Verification items for this drawing (mm, ordinates from the low corner). A direction names the side the tool comes from. Round coordinates to 2 decimals unless told otherwise and drop trailing zeros. Order: outer loops, then holes, each group sorted by start corner. A loop starts at its lowest first (then second) coordinate and runs counter-clockwise, first axis right, second up. Notation, with made-up numbers: (-35, 16.25) -> (10, 16.25) arc R18 cw to (10, 43.25) -> close; hole circle Ø4 at (59.25, 84). An arc over 180 degrees is marked (long way). Answer in a Markdown table with one row per item. Add a question column.
1. Material ranges on L1, parallel to Y at x = 14, z = 6; L2, parallel to Y at x = 13, z = 9.5; L3, parallel to Z at x = 22.5, y = 58, recorded low to high. Write a range as from..to.
2. Sectioned sample at C-C, the plane x = 35.5. Record the boundary of the cut face in (y, z).
3. Access from +Z, -Z, +X, -X, +Y, -Y to the whole of each face (thin tool, end or side, straight path). Record for the marked faces 1, 2, 3, 4 and 5.
4. Sectioned sample at A-A, the plane x = 14. Record the boundary of the cut face in (y, z), then the cut area to 3 significant figures.
5. Sectioned sample at B-B, the plane z = 5.5. Record the boundary of the cut face in (x, y), then the cut area to 3 significant figures.
6. Depth check by flat-ended pin: P1, Ø7, axis at x = 14, y = 55, coming from the -Z side; P2, Ø3.5, axis at x = 14, y = 30, coming from the -Z side; P3, Ø6, axis at y = 38.5, z = 8, coming from the +X side. Enter the tip coordinate at first touch or a pass-through.
7. Sectioned sample at D-D, the plane y = 30. Record the boundary of the cut face in (x, z), then the cut area to 3 significant figures.
8. Draft check along X on the marked faces 6, 7, 8 and 9. Enter one of: +X half, -X half, draft (parallel to the pull), parting line (faces both ways), or undercut.
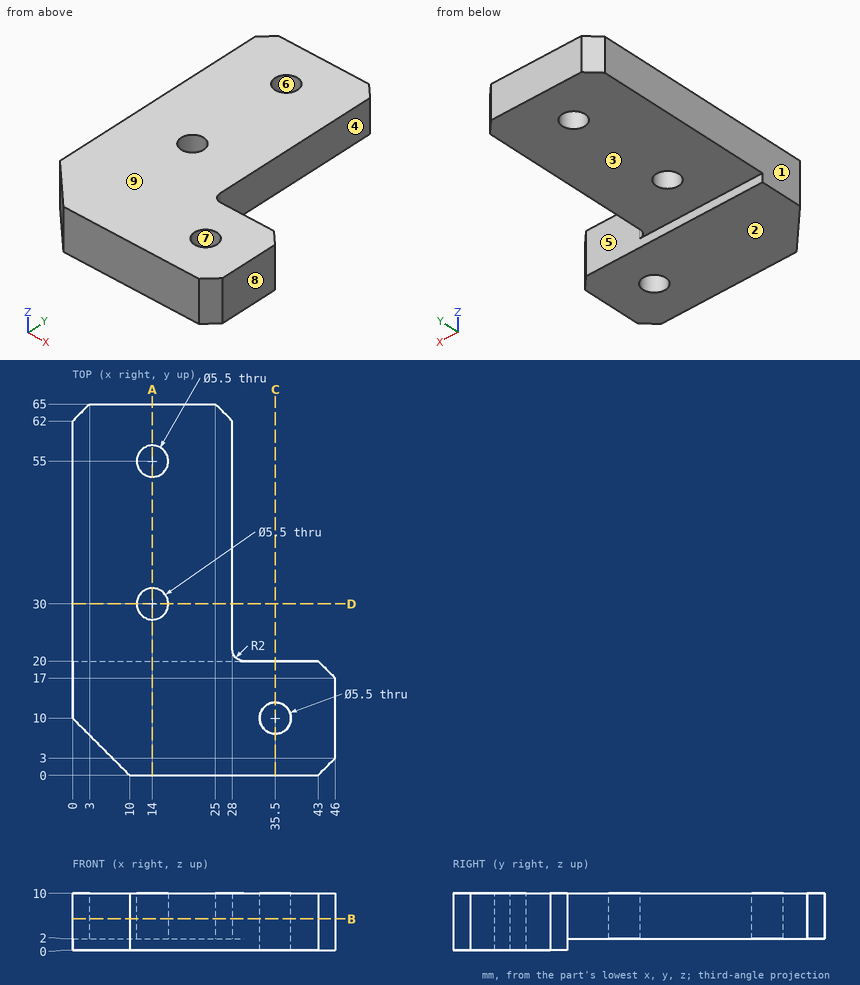
Answer key:
| question | item | result |
|---|---|---|
| 1 | L1 | y = 0..27.25, 32.75..52.25, 57.75..65 |
| 1 | L2 | y = 0..27.44, 32.56..52.44, 57.56..65 |
| 1 | L3 | z = 2..10 |
| 2 | outline | (0, 0) -> (7.25, 0) -> (7.25, 10) -> (0, 10) -> close; (12.75, 0) -> (20, 0) -> (20, 10) -> (12.75, 10) -> close |
| 3 | face 1 | +Z, -Z, -X, +Y, -Y |
| 3 | face 2 | -Z, +X, -X, +Y, -Y |
| 3 | face 3 | -Z, +X, -X, +Y |
| 3 | face 4 | +Z, -Z, +X, +Y |
| 3 | face 5 | -Z, +X, +Y |
| 4 | outline | (0, 0) -> (20, 0) -> (20, 2) -> (27.25, 2) -> (27.25, 10) -> (0, 10) -> close; (32.75, 2) -> (52.25, 2) -> (52.25, 10) -> (32.75, 10) -> close; (57.75, 2) -> (65, 2) -> (65, 10) -> (57.75, 10) -> close |
| 4 | area | 472 mm² |
| 5 | outline | (0, 10) -> (10, 0) -> (43, 0) -> (46, 3) -> (46, 17) -> (43, 20) -> (30, 20) arc R2 cw to (28, 22) -> (28, 62) -> (25, 65) -> (3, 65) -> (0, 62) -> close; hole circle Ø5.5 at (14, 30); hole circle Ø5.5 at (14, 55); hole circle Ø5.5 at (35.5, 10) |
| 5 | area | 2,040 mm² |
| 6 | P1 | stops at z = 2 |
| 6 | P2 | passes through |
| 6 | P3 | stops at x = 28 |
| 7 | outline | (0, 2) -> (11.25, 2) -> (11.25, 10) -> (0, 10) -> close; (16.75, 2) -> (28, 2) -> (28, 10) -> (16.75, 10) -> close |
| 7 | area | 180 mm² |
| 8 | face 6 | undercut |
| 8 | face 7 | undercut |
| 8 | face 8 | +X half |
| 8 | face 9 | draft |
